```python
from build123d import *

# Parameters (mm, degrees)
SKETCH_1_W          = 600
SKETCH_1_H          = 425
EXTRUDE_1_DEPTH     = 1000
SHELL_2_T           = -2
SKETCH_2_W          = 540
SKETCH_2_H          = 998
CUT_EXTRUDE_1_DEPTH = 900
SKETCH_5_W          = 28
SKETCH_5_H          = 421
EXTRUDE_2_DEPTH     = 2
SKETCH_6_W          = 120
SKETCH_6_H          = 120
CUT_EXTRUDE_3_DEPTH = 812
SKETCH_7_R          = 3
CUT_EXTRUDE_4_DEPTH = 1118
SKETCH_8_R          = 3
CUT_EXTRUDE_5_DEPTH = 671


with BuildPart() as part:
    # 草图1 → 凸台-拉伸1 (new body)
    with BuildSketch(Plane(origin=(0, 0, 0), x_dir=(1, 0, 0), z_dir=(0, 1, 0))):
        with Locations((300, 212.5)):
            Rectangle(SKETCH_1_W, SKETCH_1_H)
    extrude(amount=EXTRUDE_1_DEPTH)

    # 抽壳2
    shell_2_openings = [part.faces().sort_by_distance(p)[0] for p in [
        (300, 0, -212.5),
    ]]
    offset(amount=SHELL_2_T, openings=shell_2_openings, kind=Kind.INTERSECTION)

    # 草图2 → 切除-拉伸1 (cut)
    with BuildSketch(Plane.XY):
        with Locations((300, 499)):
            Rectangle(SKETCH_2_W, SKETCH_2_H)
    extrude(amount=-CUT_EXTRUDE_1_DEPTH, mode=Mode.SUBTRACT)

    # 草图5 → 凸台-拉伸2 (add)
    with BuildSketch(Plane.XZ):
        with Locations((16, -212.5)):
            Rectangle(SKETCH_5_W, SKETCH_5_H)
        with Locations((584, -212.5)):
            Rectangle(SKETCH_5_W, SKETCH_5_H)
    extrude(amount=-EXTRUDE_2_DEPTH)

    # 草图6 → 切除-拉伸3 (cut)
    with BuildSketch(Plane(origin=(600, 0, 0), x_dir=(0, 0, -1), z_dir=(1, 0, 0))):
        with Locations((180, 180)):
            Rectangle(SKETCH_6_W, SKETCH_6_H)
    extrude(amount=-CUT_EXTRUDE_3_DEPTH, mode=Mode.SUBTRACT)

    # 草图7 → 切除-拉伸4 (cut)
    with BuildSketch(Plane.XZ):
        with Locations(Location((15, -115, 0), (0, 0, 270))):
            Circle(SKETCH_7_R)
        with Locations(Location((585, -415, 0), (0, 0, 90))):
            Circle(SKETCH_7_R)
        with Locations(Location((15, -415, 0), (0, 0, 270))):
            Circle(SKETCH_7_R)
        with Locations(Location((585, -115, 0), (0, 0, 90))):
            Circle(SKETCH_7_R)
    extrude(amount=-CUT_EXTRUDE_4_DEPTH, mode=Mode.SUBTRACT)

    # 草图8 → 切除-拉伸5 (cut)
    with BuildSketch(Plane(origin=(0, 0, -425), x_dir=(-1, 0, 0), z_dir=(0, 0, -1))):
        with Locations((-15, 30)):
            Circle(SKETCH_8_R)
        with Locations((-15, 330)):
            Circle(SKETCH_8_R)
        with Locations((-15, 630)):
            Circle(SKETCH_8_R)
        with Locations(Location((-585, 30, 0), (0, 0, 180))):
            Circle(SKETCH_8_R)
        with Locations(Location((-585, 330, 0), (0, 0, 180))):
            Circle(SKETCH_8_R)
        with Locations((-15, 880)):
            Circle(SKETCH_8_R)
        with Locations(Location((-585, 630, 0), (0, 0, 180))):
            Circle(SKETCH_8_R)
        with Locations(Location((-585, 880, 0), (0, 0, 180))):
            Circle(SKETCH_8_R)
    extrude(amount=-CUT_EXTRUDE_5_DEPTH, mode=Mode.SUBTRACT)


solid = part.part
```
Model file for the job. Use its own axes, mm. A direction names the side the tool comes from. Round coordinates to 2 decimals unless told otherwise and drop trailing zeros. Order: outer loops, then holes, each group sorted by start corner. A loop starts at its lowest first (then second) coordinate and runs counter-clockwise, first axis right, second up. Notation, with made-up numbers: (-19, 68) -> (26, 68) arc R21 cw to (26, 101) -> close; hole circle Ø6 at (26, 88.25). An arc over 180 degrees is marked (long way). Use one line per item in the form item = value.
Item 1: Cut at C-C, the plane x = 243. Write the cut outline in (y, z), and give its area (3 significant figures).
Returned:
outline = (998, -425) -> (1000, -425) -> (1000, 0) -> (998, 0) -> close
area = 850 mm^2
Item 2: Flat gauge pins, fed straight in: pin 1 Ø5 at (x, z) = (15, -115) entering from +Y; pin 2 Ø8 at (x, z) = (352.5, -264.5) entering from -Y. Where does each tip first touch, or does it go through?
Returned:
pin_1 = through
pin_2 = 998
Item 3: Drill centre lines: line 1 (Y direction, x = 585, z = -1.05); line 2 (X direction, y = 880, z = -0.75); line 3 (X direction, y = 999.3, z = -115). Where is each one in solid material? Low to high.
Returned:
line_1 = 0 to 27, 33 to 327, 333 to 627, 633 to 877, 883 to 1000
line_2 = 0 to 12, 18 to 30, 570 to 582, 588 to 600
line_3 = 0 to 12, 18 to 582, 588 to 600
Item 4: Cut at A-A, the plane y = 380. Write the cut outline in (x, z).
Returned:
outline = (0, -425) -> (30, -425) -> (30, -423) -> (2, -423) -> (2, -2) -> (30, -2) -> (30, 0) -> (0, 0) -> close; (570, -425) -> (600, -425) -> (600, 0) -> (570, 0) -> (570, -2) -> (598, -2) -> (598, -423) -> (570, -423) -> close
Item 5: Pull direction Z, two halves, no side cores. Call faces 3 (the face through (587, 498, 0)), 4 (the face through (2, 493, -210)), 5 (the face through (585, 0, -215)): released by +Z, released by -Z, zero draft, split by the parting line, or undercut.
Returned:
face_3 = released by +Z
face_4 = undercut
face_5 = zero draft
Item 6: Cut at B-B, the plane z = -397. Write the cut outline in (x, y).
Returned:
outline = (0, 0) -> (30, 0) -> (30, 2) -> (2, 2) -> (2, 998) -> (598, 998) -> (598, 2) -> (570, 2) -> (570, 0) -> (600, 0) -> (600, 1000) -> (0, 1000) -> close
Item 7: Tool access for faces 1 (the face through (0, 493, -210)), 2 (the face through (16, 493, -423)): list every direction of +Z, -Z, +X, -X, +Y, -Y with a clear straight run to the whole face (end or side of a thin tool).
Returned:
face_1 = +Z, -Z, -X, +Y, -Y
face_2 = none
